Source: CAD feature listing. Evaluate the final solid. Frame: model axes, mm. A direction names the side the tool comes from. Give positions to 0.01 mm unless a question says otherwise; leave off trailing zeros. Order: outer loops, then holes, each group sorted by start corner. A loop starts at its lowest first (then second) coordinate and runs counter-clockwise, first axis right, second up. Notation, with made-up numbers: (46.5, -12.5) -> (69.5, -12.5) arc R24 cw to (69.5, 12.5) -> close; hole circle Ø3 at (44.25, 51). An arc over 180 degrees is marked (long way). Use CSV: the item, a comma, the result in double quotes.
```python
from build123d import *

# Parameters (mm, degrees)
BASE_PLATE_SKETCH_W         = 100
BASE_PLATE_SKETCH_H         = 50
BASE_PLATE_100X50X10_DEPTH  = 10
OVAL_BOSS_DEPTH             = 40
SUPPORT_RIB_1_REACH         = 116.564
SUPPORT_RIB_1_SKETCH_WALL_W = 284.279513812
SUPPORT_RIB_1_SKETCH_WALL_H = 10
SUPPORT_RIB_2_REACH         = 116.564
SUPPORT_RIB_2_SKETCH_WALL_W = 284.279513812
SUPPORT_RIB_2_SKETCH_WALL_H = 10
RAISED_PADS_SKETCH_R        = 7
RAISED_PADS_SKETCH_R_2      = 6
RAISED_PADS_2MM_DEPTH       = 2
MOUNTING_HOLE_1_SKETCH_R    = 6
MOUNTING_HOLE_1_DEPTH       = 119.74342087
MOUNTING_HOLE_2_SKETCH_R    = 6
MOUNTING_HOLE_2_DEPTH       = 119.74342087
MOUNTING_HOLE_3_SKETCH_R    = 6
MOUNTING_HOLE_3_DEPTH       = 119.084715353
MOUNTING_HOLE_4_SKETCH_R    = 6
MOUNTING_HOLE_4_DEPTH       = 119.74342087
BOSS_BORE_DEPTH             = 119.74342087


with BuildPart() as part:
    # Base Plate Sketch → Base Plate 100x50x10 (new body)
    with BuildSketch(Plane.XY):
        with Locations((50, 25)):
            Rectangle(BASE_PLATE_SKETCH_W, BASE_PLATE_SKETCH_H)
    extrude(amount=BASE_PLATE_100X50X10_DEPTH)

    # Oval Boss Sketch → Oval Boss (add)
    with BuildSketch(Plane.XY.offset(10)):
        with BuildLine():
            Line((35, 15), (35, 35))
            ThreePointArc((35, 35), (50, 50), (65, 35))
            Line((65, 35), (65, 15))
            ThreePointArc((65, 15), (50, 0), (35, 15))
        make_face()
        with BuildLine():
            Line((40, 15), (40, 35))
            ThreePointArc((40, 35), (50, 45), (60, 35))
            Line((60, 35), (60, 15))
            ThreePointArc((60, 15), (50, 5), (40, 15))
        make_face(mode=Mode.SUBTRACT)
    extrude(amount=OVAL_BOSS_DEPTH)

    # Support Rib 1 Sketch wall → Support Rib 1 (add, up to next)
    with BuildSketch(Plane(origin=(82.5, 25, 30), x_dir=(0.658504607869, 0, -0.752576694707), z_dir=(-0.752576694707, 0, -0.658504607869)), mode=Mode.PRIVATE) as support_rib_1_sk1:
        Rectangle(SUPPORT_RIB_1_SKETCH_WALL_W, SUPPORT_RIB_1_SKETCH_WALL_H)
    support_rib_1_tool1 = extrude(support_rib_1_sk1.sketch, amount=SUPPORT_RIB_1_REACH, mode=Mode.PRIVATE) - part.part
    add(support_rib_1_tool1.solids().sort_by_distance((82.5, 25, 30))[0])

    # Support Rib 2 Sketch wall → Support Rib 2 (add, up to next)
    with BuildSketch(Plane(origin=(17.5, 25, 30), x_dir=(-0.658504607869, 0, -0.752576694707), z_dir=(-0.752576694707, 0, 0.658504607869)), mode=Mode.PRIVATE) as support_rib_2_sk1:
        Rectangle(SUPPORT_RIB_2_SKETCH_WALL_W, SUPPORT_RIB_2_SKETCH_WALL_H)
    support_rib_2_tool1 = extrude(support_rib_2_sk1.sketch, amount=-SUPPORT_RIB_2_REACH, mode=Mode.PRIVATE) - part.part
    add(support_rib_2_tool1.solids().sort_by_distance((17.5, 25, 30))[0])

    # Raised Pads Sketch → Raised Pads 2mm (add)
    # profile 1 of 4: a face of its own
    with BuildSketch(Plane.XY.offset(10)):
        with Locations((17.5, 10)):
            Circle(RAISED_PADS_SKETCH_R)
        with Locations((17.5, 10)):
            Circle(RAISED_PADS_SKETCH_R_2, mode=Mode.SUBTRACT)
    # profile 2 of 4: a face of its own
    with BuildSketch(Plane.XY.offset(10)):
        with Locations((82.5, 10)):
            Circle(RAISED_PADS_SKETCH_R)
        with Locations((82.5, 10)):
            Circle(RAISED_PADS_SKETCH_R_2, mode=Mode.SUBTRACT)
    # profile 3 of 4: a face of its own
    with BuildSketch(Plane.XY.offset(10)):
        with Locations((17.5, 40)):
            Circle(RAISED_PADS_SKETCH_R)
        with Locations((17.5, 40)):
            Circle(RAISED_PADS_SKETCH_R_2, mode=Mode.SUBTRACT)
    # profile 4 of 4: a face of its own
    with BuildSketch(Plane.XY.offset(10)):
        with Locations((82.5, 40)):
            Circle(RAISED_PADS_SKETCH_R_2)
    extrude(amount=RAISED_PADS_2MM_DEPTH)

    # Mounting Hole 1 Sketch → Mounting Hole 1 (cut, through all)
    with BuildSketch(Plane.XY.offset(10)):
        with Locations((17.5, 40)):
            Circle(MOUNTING_HOLE_1_SKETCH_R)
    extrude(amount=-MOUNTING_HOLE_1_DEPTH, mode=Mode.SUBTRACT)

    # Mounting Hole 2 Sketch → Mounting Hole 2 (cut, through all)
    with BuildSketch(Plane.XY.offset(10)):
        with Locations((17.5, 10)):
            Circle(MOUNTING_HOLE_2_SKETCH_R)
    extrude(amount=-MOUNTING_HOLE_2_DEPTH, mode=Mode.SUBTRACT)

    # Mounting Hole 3 Sketch → Mounting Hole 3 (cut, through all)
    with BuildSketch(Plane.XY.offset(12)):
        with Locations((82.5, 40)):
            Circle(MOUNTING_HOLE_3_SKETCH_R)
    extrude(amount=-MOUNTING_HOLE_3_DEPTH, mode=Mode.SUBTRACT)

    # Mounting Hole 4 Sketch → Mounting Hole 4 (cut, through all)
    with BuildSketch(Plane.XY.offset(10)):
        with Locations((82.5, 10)):
            Circle(MOUNTING_HOLE_4_SKETCH_R)
    extrude(amount=-MOUNTING_HOLE_4_DEPTH, mode=Mode.SUBTRACT)

    # Boss Bore Sketch → Boss Bore (cut, through all)
    with BuildSketch(Plane.XY.offset(10)):
        with BuildLine():
            Line((39.934647115, 15), (39.934647115, 35))
            ThreePointArc((39.934647115, 35), (50, 45.065352885), (60.065352885, 35))
            Line((60.065352885, 35), (60.065352885, 15))
            ThreePointArc((60.065352885, 15), (50, 4.934647115), (39.934647115, 15))
        make_face()
    extrude(amount=-BOSS_BORE_DEPTH, mode=Mode.SUBTRACT)


solid = part.part
```
1. Ray query, line 1 along Y through (x, z) = (17.5, 3.25); line 2 along Y through (x, z) = (17.5, 10.7); line 3 along X through (y, z) = (28, 4.5). Return the intervals inside material, ascending.
Answer below:
line 1,"y = 0 to 4, 16 to 34, 46 to 50"
line 2,"y = 3 to 4, 16 to 17, 20 to 30, 33 to 34, 46 to 47"
line 3,"x = 0 to 39.93, 60.07 to 100"
2. Pin query (flat end, axial travel): P1, Ø2, axis at x = 15, z = 28, coming from the +Y side; P2, Ø1.5, axis at y = 18, z = 36.5, coming from the +X side; P3, Ø1.5, axis at x = 74.5, y = 22.5, coming from the +Z side. Return the tip coordinate at first contact, or that it passes through.
Answer below:
P1,"stops at y = 30"
P2,"stops at x = 65"
P3,"stops at z = 40"
3. Mould query, pull axis X, two halves, no side actions, for faces 1 (the flat face through (23, 13, 12)), 2 (the flat face through (60.065, 25, 5)), 3 (the flat face through (17.745, 24.93, 30.28)). Classes: released by +X, released by -X, zero draft, split by the parting line, or undercut.
Answer below:
face 1,"zero draft"
face 2,"undercut"
face 3,"released by -X"
4. Section query A-A on z = 40. Return loops of the section in (x, y), plus the area to 3 significant figures.
Answer below:
outline,"(26.25, 20) -> (35, 20) -> (35, 15) arc R15 ccw to (65, 15) -> (65, 20) -> (73.75, 20) -> (73.75, 30) -> (65, 30) -> (65, 35) arc R15 ccw to (35, 35) -> (35, 30) -> (26.25, 30) -> close; hole (40, 15) arc R10 ccw to (60, 15) -> (60, 35) arc R10 ccw to (40, 35) -> close"
area,"768 mm²"
5. Section query D-D on z = 8. Return loops of the section in (x, y).
Answer below:
outline,"(0, 0) -> (100, 0) -> (100, 50) -> (0, 50) -> close; hole circle Ø12 at (17.5, 10); hole circle Ø12 at (17.5, 40); hole (39.93, 15) arc R10.07 ccw to (60.07, 15) -> (60.07, 35) arc R10.07 ccw to (39.93, 35) -> close; hole circle Ø12 at (82.5, 10); hole circle Ø12 at (82.5, 40)"
6. Section query C-C on x = 82.5. Return loops of the section in (y, z).
Answer below:
outline,"(0, 0) -> (4, 0) -> (4, 12) -> (3, 12) -> (3, 10) -> (0, 10) -> close; (16, 0) -> (34, 0) -> (34, 10) -> (30, 10) -> (30, 30) -> (20, 30) -> (20, 10) -> (17, 10) -> (17, 12) -> (16, 12) -> close; (46, 0) -> (50, 0) -> (50, 10) -> (46, 10) -> close"
7. Section query B-B on y = 21. Return loops of the section in (x, z), plus the area to 3 significant figures.
Answer below:
outline,"(0, 0) -> (39.93, 0) -> (39.93, 10) -> (40, 10) -> (40, 50) -> (35, 50) -> (0, 10) -> close; (60, 10) -> (60.07, 10) -> (60.07, 0) -> (100, 0) -> (100, 10) -> (65, 50) -> (60, 50) -> close"
area,"2,600 mm²"
8. Access query for faces 4 (the flat face through (80, 47, 10)), 5 (the cylindrical face through (75.507, 10.308, 10.986)), 6 (the cylindrical face through (50, 45, 30)), 7 (the flat face through (88, 13, 12)), 8 (the flat face through (0, 25, 5)). Directions: +Z, -Z, +X, -X, +Y, -Y. A direction counts if a zero-diameter tool reaches every point of the face in a straight line with its end or side. Return the directions, or none.
Answer below:
face 4,"+Z, +X, +Y"
face 5,"+Z"
face 6,"+Z, -Z"
face 7,"+Z, +X, -Y"
face 8,"+Z, -Z, -X, +Y, -Y"
